```python
from build123d import *

# Parameters (mm, degrees)
SKETCH_1_W          = 72
SKETCH_1_H          = 13
EXTRUDE_1_DEPTH     = 39
FILLET_1_R          = 0.5
SKETCH_2_R          = 2.25
CUT_EXTRUDE_1_DEPTH = 55.644304369


with BuildPart() as part:
    # 草图1 → 凸台-拉伸1 (new body)
    with BuildSketch(Plane.XY):
        Rectangle(SKETCH_1_W, SKETCH_1_H)
    extrude(amount=EXTRUDE_1_DEPTH)

    # 圆角1
    fillet_1_edges = [part.edges().sort_by_distance(p)[0] for p in [
        (36, 0, 39),
        (-36, 0, 39),
        (36, 0, 0),
        (-36, 0, 0),
    ]]
    fillet(fillet_1_edges, radius=FILLET_1_R)

    # 草图2 → 切除-拉伸1 (cut, through all)
    with BuildSketch(Plane(origin=(0, 6.5, 0), x_dir=(1, 0, 0), z_dir=(0, 1, 0))):
        with Locations(Location((-20, -28.5, 0), (0, 0, 180))):
            Circle(SKETCH_2_R)
        with Locations(Location((20, -28.5, 0), (0, 0, 180))):
            Circle(SKETCH_2_R)
    extrude(amount=-CUT_EXTRUDE_1_DEPTH, mode=Mode.SUBTRACT)


solid = part.part
```
For this review, take the finished solid that the model builds, in its own axes (mm). Coordinates: 2 decimals unless noted, no trailing zeros. Order: outer loops, then holes, each group sorted by start corner. A loop starts at its lowest first (then second) coordinate and runs counter-clockwise, first axis right, second up. Notation, with made-up numbers: (82.25, 16) -> (86.25, 16) arc R21 cw to (86.25, 29) -> close; hole circle Ø2 at (-29, -35.75). An arc over 180 degrees is marked (long way). Answer as CSV lines item,"result".
Q1. We need section B-B (x = -20). State the section outline as (y, z) points, plus the area to 4 significant figures.
Model answer:
outline,"(-6.5, 0) -> (6.5, 0) -> (6.5, 26.25) -> (-6.5, 26.25) -> close; (-6.5, 30.75) -> (6.5, 30.75) -> (6.5, 39) -> (-6.5, 39) -> close"
area,"448.5 mm2"
Q2. Draft analysis for pull direction X (two halves, no side actions). For faces 1 (the face through (0, 0, 39)), 2 (the face through (-21.038, 0.091, 26.504)), 3 (the face through (-36, 0, 19)), state which applies: released by +X, released by -X, zero draft, split by the parting line, or undercut.
Model answer:
face 1,"zero draft"
face 2,"undercut"
face 3,"released by -X"
Q3. We need section A-A (z = 28.5). State the section outline as (x, y) points.
Model answer:
outline,"(-36, -6.5) -> (-22.25, -6.5) -> (-22.25, 6.5) -> (-36, 6.5) -> close; (-17.75, -6.5) -> (17.75, -6.5) -> (17.75, 6.5) -> (-17.75, 6.5) -> close; (22.25, -6.5) -> (36, -6.5) -> (36, 6.5) -> (22.25, 6.5) -> close"
Q4. Clearance check with a flat-ended pin moving along its axis: pin 1 Ø3.5 at (x, z) = (-20, 28.5) entering from -Y. State where the tip first meets the part, or that it passes through.
Model answer:
pin 1,"passes through"
Q5. Wall thickness on line 1 along Z through (x, y) = (-20, -2.5); line 2 along Z through (x, y) = (-21, -0.25): over which ranges is each line inside the solid? List them lowest first. Write a range as [from, to].
Model answer:
line 1,"z = [0, 26.25], [30.75, 39]"
line 2,"z = [0, 26.48], [30.52, 39]"
